Part model, mm, in its own coordinate system. A direction names the side the tool comes from. Give positions to 0.01 mm unless a question says otherwise; leave off trailing zeros. Write each loop counter-clockwise with the first axis right and the second up, starting at its lowest first coordinate (ties: lowest second). Pieces come first, ordered by that corner, then holes. Notation, with made-up numbers: M 54,38 L 63,38 A15 ccw 63,49 Z; hole C 77.5,36.25 d8. An arc over 180 degrees is marked long. Use a Markdown table: item, result. Add a question column.
from build123d import *

# Parameters (mm, degrees)
SKETCH_1_W      = 400
SKETCH_1_H      = 250
EXTRUDE_1_DEPTH = 350
SHELL_1_T       = -5
SKETCH_2_W      = 150
SKETCH_2_H      = 60
EXTRUDE_2_DEPTH = 5
SKETCH_3_W      = 150
SKETCH_3_H      = 60
EXTRUDE_3_DEPTH = 5


with BuildPart() as part:
    # 草图1 → 凸台-拉伸1 (new body)
    with BuildSketch(Plane(origin=(0, 0, 0), x_dir=(1, 0, 0), z_dir=(0, 1, 0))):
        with Locations((200, 125)):
            Rectangle(SKETCH_1_W, SKETCH_1_H)
    extrude(amount=EXTRUDE_1_DEPTH)

    # 抽壳1
    shell_1_openings = [part.faces().sort_by_distance(p)[0] for p in [
        (200, 350, -125),
    ]]
    offset(amount=SHELL_1_T, openings=shell_1_openings, kind=Kind.INTERSECTION)

    # 草图2 → 凸台-拉伸2 (add)
    with BuildSketch(Plane(origin=(400, 0, 0), x_dir=(0, 0, -1), z_dir=(1, 0, 0))):
        with Locations((125, 300)):
            Rectangle(SKETCH_2_W, SKETCH_2_H)
    extrude(amount=EXTRUDE_2_DEPTH)

    # 草图3 → 凸台-拉伸3 (add)
    with BuildSketch(Plane.ZY):
        with Locations((-125, 300)):
            Rectangle(SKETCH_3_W, SKETCH_3_H)
    extrude(amount=EXTRUDE_3_DEPTH)


solid = part.part
1. Cut at B-B (y = 165). Write the cut outline in (x, z).
2. Cut at A-A (x = 137). Write the cut outline in (y, z), then the cut area to 3 significant figures.
3. Mould opens along Z. For faces 1 (the flat face through (197, 173, 0)), 2 (the flat face through (-5, 300, -126)), 3 (the flat face through (197, 175, -5)) say: released by +Z, released by -Z, zero draft, split by the parting line, or undercut.
4. Drill centre lines: probe 1 along Z at (x, y) = (260, 85); probe 2 along X at (y, z) = (300, -180.5); probe 3 along X at (y, z) = (265, -237.5). Where is each one in solid material? Low to high. Write a range as [from, to].
5. Cut at C-C (z = -38.5). Write the cut outline in (x, y), then the cut area to 3 significant figures.
6. Tool access for faces 4 (the flat face through (5, 175, -123)), 5 (the flat face through (199, 350, -246)): list every direction of +Z, -Z, +X, -X, +Y, -Y with a clear straight run to the whole face (end or side of a thin tool).
7. Flat gauge pins, fed straight in: pin 1 (4 mm diameter, centred on x = -3, z = -88, fed in from +Y); pin 2 (12 mm diameter, centred on x = 245, z = -223, fed in from +Y); pin 3 (12 mm diameter, centred on y = 45.5, z = -114.5, fed in from -X). Where does each tip first touch, or does it go through?
8. Cut at D-D (z = -156). Write the cut outline in (x, y), then the cut area to 3 significant figures.
A:
| question | item | result |
|---|---|---|
| 1 | outline | M 0,-250 L 400,-250 L 400,0 L 0,0 Z; hole M 5,-245 L 395,-245 L 395,-5 L 5,-5 Z |
| 2 | outline | M 0,-250 L 350,-250 L 350,-245 L 5,-245 L 5,-5 L 350,-5 L 350,0 L 0,0 Z |
| 2 | area | 4,700 mm² |
| 3 | face 1 | released by +Z |
| 3 | face 2 | zero draft |
| 3 | face 3 | undercut |
| 4 | probe 1 | z = [-250, -245], [-5, 0] |
| 4 | probe 2 | x = [-5, 5], [395, 405] |
| 4 | probe 3 | x = [0, 5], [395, 400] |
| 5 | outline | M 0,0 L 400,0 L 400,350 L 395,350 L 395,5 L 5,5 L 5,350 L 0,350 Z |
| 5 | area | 5,450 mm² |
| 6 | face 4 | +Y |
| 6 | face 5 | +Z, -Z, +X, -X, +Y |
| 7 | pin 1 | stops at y = 330 |
| 7 | pin 2 | stops at y = 5 |
| 7 | pin 3 | stops at x = 0 |
| 8 | outline | M -5,270 L 0,270 L 0,0 L 400,0 L 400,270 L 405,270 L 405,330 L 400,330 L 400,350 L 395,350 L 395,5 L 5,5 L 5,350 L 0,350 L 0,330 L -5,330 Z |
| 8 | area | 6,050 mm² |
